Verification items for this drawing (mm, ordinates from the low corner). Round coordinates to 2 decimals unless told otherwise and drop trailing zeros. Order: outer loops, then holes, each group sorted by start corner. A loop starts at its lowest first (then second) coordinate and runs counter-clockwise, first axis right, second up. Notation, with made-up numbers: (-19.75, -5.75) - (38.25, -5.75) arc R34 ccw to (38.25, 29.25) - close; hole circle Ø10 at (51, 9.25). An arc over 180 degrees is marked (long way). Use a Markdown table: item, result. Add a question column.
(1) Section check A-A on y = 75. Record the boundary of the cut face in (x, z).
(2) Thickness scan on line 1 along Y through (x, z) = (26, 12.5); line 2 along X through (y, z) = (69.5, 20.5); line 3 along Y through (x, z) = (14.5, 17.75). Record the ranges inside material, lowest first. Write a range as [from, to].
(3) Gauge pin test, flat ends, axial feed: P1, Ø4, axis at x = 15, z = 21, coming from the +Y side; P2, Ø1, axis at y = 40, z = 18.5, coming from the +X side. Record the tip position at first contact, or that the pin passes through.
(4) Section check B-B on x = 71.5. Record the boundary of the cut face in (y, z), then the cut area to 3 significant figures.
(5) Section check C-C on z = 19.25. Record the boundary of the cut face in (x, y).
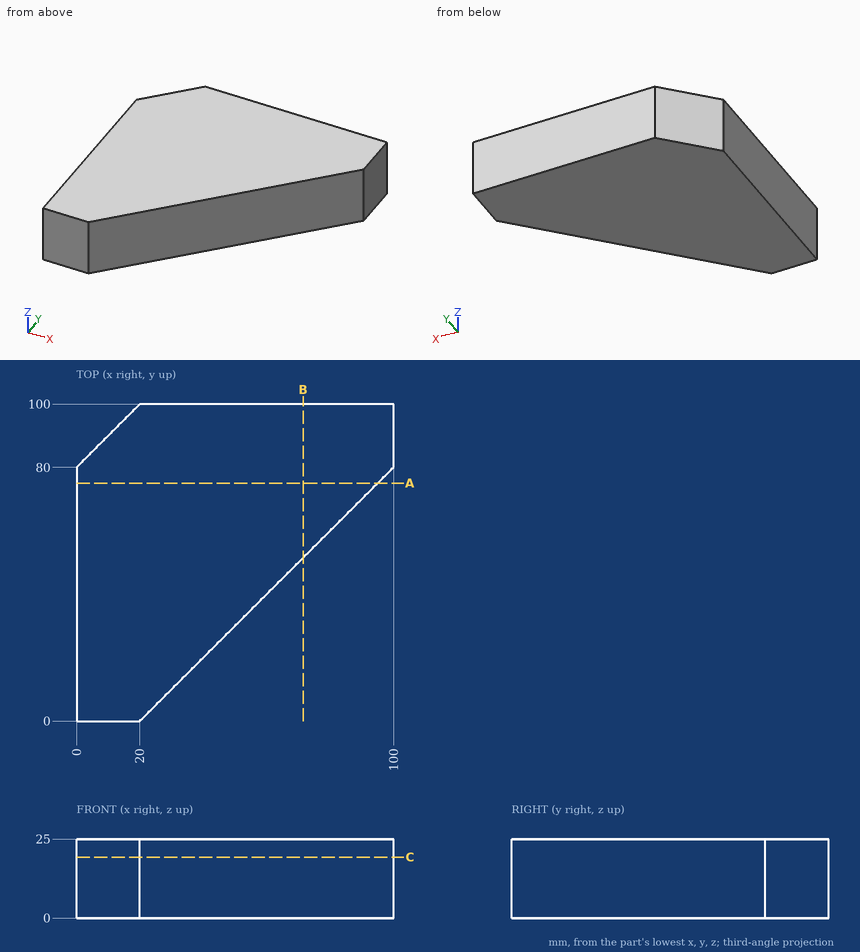
Check sheet entries:
| question | item | result |
|---|---|---|
| 1 | outline | (0, 0) - (95, 0) - (95, 25) - (0, 25) - close |
| 2 | line 1 | y = [6, 100] |
| 2 | line 2 | x = [0, 89.5] |
| 2 | line 3 | y = [0, 94.5] |
| 3 | P1 | stops at y = 97 |
| 3 | P2 | stops at x = 60.5 |
| 4 | outline | (51.5, 0) - (100, 0) - (100, 25) - (51.5, 25) - close |
| 4 | area | 1,210 mm2 |
| 5 | outline | (0, 0) - (20, 0) - (100, 80) - (100, 100) - (20, 100) - (0, 80) - close |
